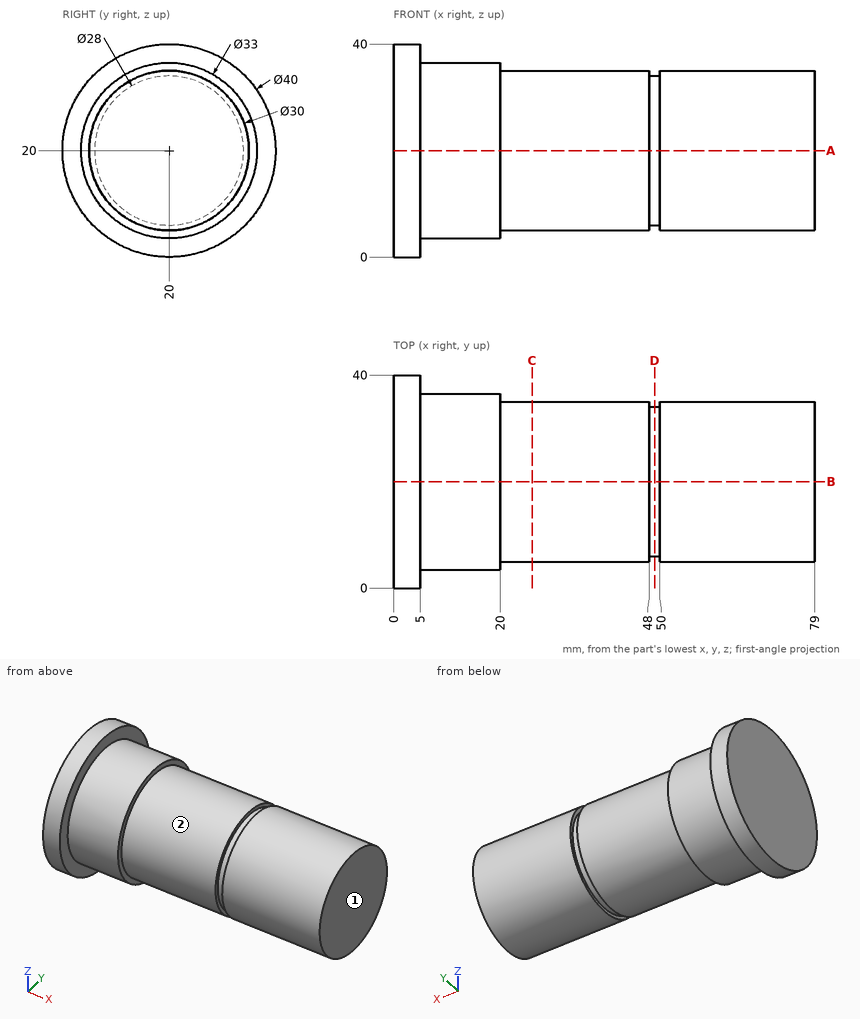
Geometry check sheet. Reference: drawing and pictorial views, mm from the part's lowest x, y, z. A direction names the side the tool comes from. Round coordinates to 2 decimals unless told otherwise and drop trailing zeros. Write each loop counter-clockwise with the first axis right and the second up, starting at its lowest first coordinate (ties: lowest second). Pieces come first, ordered by that corner, then holes. Notation, with made-up numbers: (57, -1) -> (100, -1) arc R19 ccw to (100, 4) -> close; hole circle Ø7 at (63.5, 27). An arc over 180 degrees is marked (long way). Put each result on its own line as item: value.
1) Cross-section at C-C, the plane x = 26. Enter the section's corners in (y, z), plus the area to 3 significant figures.
Recorded:
outline: circle Ø30 at (20, 20)
area: 707 mm2
2) Access from +Z, -Z, +X, -X, +Y, -Y to the whole of each face (thin tool, end or side, straight path). Record for the marked faces 1 and 2.
Recorded:
face 1: +Z, -Z, +X, +Y, -Y
face 2: +X
3) Depth check by flat-ended pin: P1, Ø12, axis at x = 15.5, y = 23.5, coming from the +Z side; P2, Ø4, axis at x = 57, z = 34, coming from the +Y side; P3, Ø5, axis at x = 28.5, y = 25.5, coming from the +Z side. Enter the tip coordinate at first touch or a pass-through.
Recorded:
P1: stops at z = 36.5
P2: stops at y = 29
P3: stops at z = 34.7
4) Cross-section at D-D, the plane x = 49. Enter the section's corners in (y, z), plus the area to 3 significant figures.
Recorded:
outline: circle Ø28 at (20, 20)
area: 616 mm2
5) Thickness scan on probe 1 along Z at (x, y) = (63, 20); probe 2 along X at (y, z) = (8, 31); probe 3 along Y at (x, z) = (51, 19.5). Record the ranges inside material, lowest first. Write a range as from..to.
Recorded:
probe 1: z = 5..35
probe 2: x = 0..20
probe 3: y = 5.01..34.99
6) Cross-section at A-A, the plane z = 20. Enter the section's corners in (x, y).
Recorded:
outline: (0, 0) -> (5, 0) -> (5, 3.5) -> (20, 3.5) -> (20, 5) -> (48, 5) -> (48, 6) -> (50, 6) -> (50, 5) -> (79, 5) -> (79, 35) -> (50, 35) -> (50, 34) -> (48, 34) -> (48, 35) -> (20, 35) -> (20, 36.5) -> (5, 36.5) -> (5, 40) -> (0, 40) -> close
